Check sheet for the modelled part. Datum: model origin and axes. Units: mm. Face numbers are marked on the shaded views. Coordinates: 2 decimals unless noted, no trailing zeros. Loops run counter-clockwise (first coordinate to the right, second up) from the corner with the lowest first, then second, coordinate; pieces in that order, holes last. Notation, with made-up numbers: (-17, 53) -> (6, 53) arc R11 ccw to (6, 69) -> close; hole circle Ø4 at (44, 58). An arc over 180 degrees is marked (long way). Use CSV: the item, a comma, the result in double quotes.
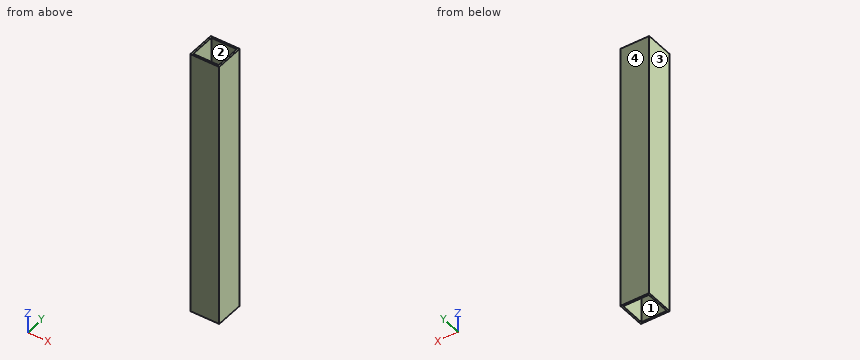
```python
from build123d import *

# Parameters (mm, degrees)
SKETCH_1_W      = 50
SKETCH_1_H      = 50
SKETCH_1_W_2    = 44
SKETCH_1_H_2    = 44
EXTRUDE_1_DEPTH = 465


with BuildPart() as part:
    # 草图1 → 凸台-拉伸1 (new body)
    with BuildSketch(Plane.XY):
        with Locations((25, 25)):
            Rectangle(SKETCH_1_W, SKETCH_1_H)
        with Locations((25, 25)):
            Rectangle(SKETCH_1_W_2, SKETCH_1_H_2, mode=Mode.SUBTRACT)
    extrude(amount=EXTRUDE_1_DEPTH)


solid = part.part
```
1) Draft check along X on the marked faces 1, 2, 3 and 4. Enter one of: released by +X, released by -X, zero draft, split by the parting line, or undercut.
Answer below:
face 1,"undercut"
face 2,"undercut"
face 3,"released by -X"
face 4,"zero draft"
2) Cross-section at C-C on z = 409. Record the boundary of the cut face in (x, y).
Answer below:
outline,"(0, 0) -> (50, 0) -> (50, 50) -> (0, 50) -> close; hole (3, 3) -> (47, 3) -> (47, 47) -> (3, 47) -> close"
3) Thickness scan on line 1 along Y through (x, z) = (8, 123.5). Record the ranges inside material, lowest first. Write a range as from..to.
Answer below:
line 1,"y = 0..3, 47..50"
4) Cross-section at A-A on x = 42.5. Record the boundary of the cut face in (y, z), and give its area (3 significant figures).
Answer below:
outline,"(0, 0) -> (3, 0) -> (3, 465) -> (0, 465) -> close; (47, 0) -> (50, 0) -> (50, 465) -> (47, 465) -> close"
area,"2,790 mm²"
